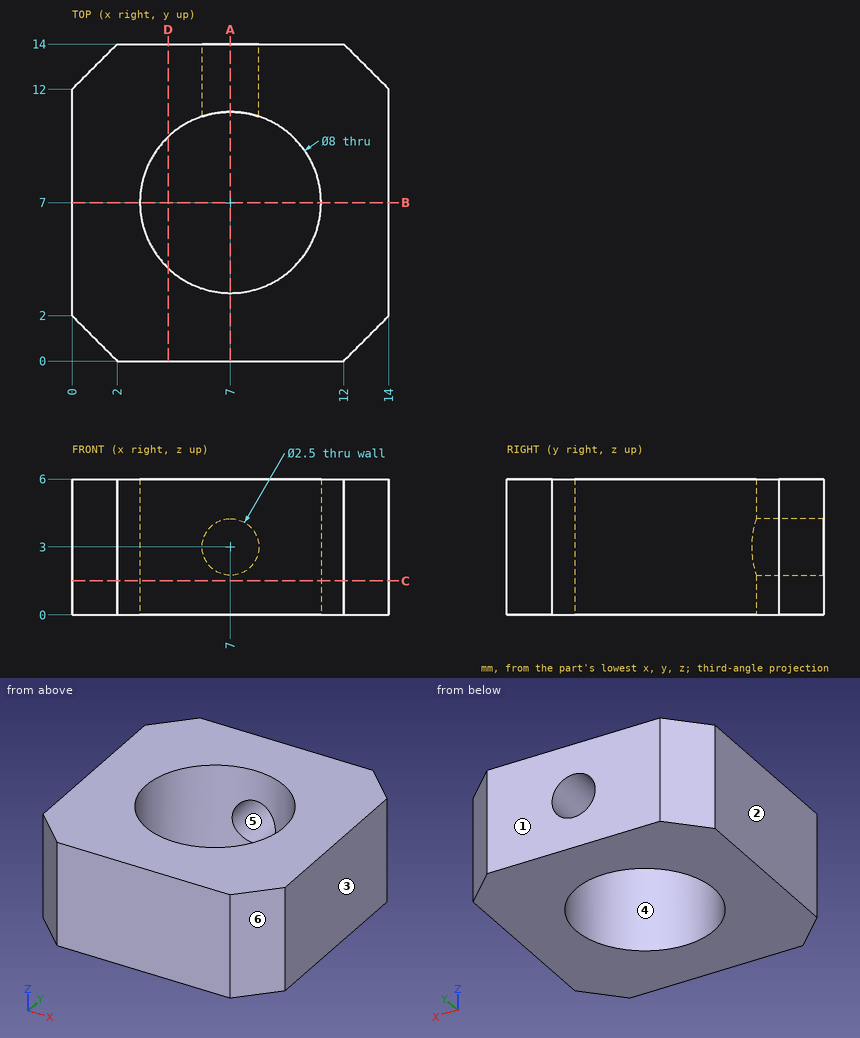
The drawing under review shows one solid part. Ordinate dimensions are in mm from its lowest x, y, z. A direction names the side the tool comes from. Coordinates: 2 decimals unless noted, no trailing zeros. Order: outer loops, then holes, each group sorted by start corner. A loop starts at its lowest first (then second) coordinate and runs counter-clockwise, first axis right, second up. Notation, with made-up numbers: (14.5, 40.25) -> (38.5, 40.25) arc R18 cw to (38.5, 68.25) -> close; hole circle Ø9 at (71.25, -14). An arc over 180 degrees is marked (long way). Answer in a Markdown table with one row per item. Add a question column.
Item 1: Mouldability with a two-part tool opening along X and no side actions: class the marked faces 1, 2, 3 and 4 as +X half, -X half, draft (parallel to the pull), parting line (faces both ways), or undercut.
Item 2: We need section D-D on x = 4.25. Write out the cut boundary in (y, z), plus the area to 3 significant figures.
Item 3: Clearance check with a flat-ended pin moving along its axis: pin 1 (2 mm diameter, centred on x = 9.5, z = 2.5, fed in from -Y). State where the tip first meets the part, or that it passes through.
Item 4: We need section B-B on y = 7. Write out the cut boundary in (x, z).
Item 5: We need section C-C on z = 1.5. Write out the cut boundary in (x, y).
Item 6: Machinability: for the marked faces 5 and 6, which of the approach directions +Z, -Z, +X, -X, +Y, -Y give a long, thin tool a straight path to every point of the face, cutting with its end or side? Answer none if there is none.
Item 7: To check wall thickness, follow probe 1 along Z at (x, y) = (7, 13.3); probe 2 along Y at (x, z) = (7, 1.5); probe 3 along X at (y, z) = (4.5, 5.25). State the ranges of each line that lie inside material, in increasing order.
Item 8: We need section A-A on x = 7. Write out the cut boundary in (y, z), plus the area to 3 significant figures.
Final values:
| question | item | result |
|---|---|---|
| 1 | face 1 | draft |
| 1 | face 2 | -X half |
| 1 | face 3 | +X half |
| 1 | face 4 | undercut |
| 2 | outline | (0, 0) -> (4.1, 0) -> (4.1, 6) -> (0, 6) -> close; (9.9, 0) -> (14, 0) -> (14, 6) -> (9.9, 6) -> close |
| 2 | area | 49.1 mm2 |
| 3 | pin 1 | stops at y = 0 |
| 4 | outline | (0, 0) -> (3, 0) -> (3, 6) -> (0, 6) -> close; (11, 0) -> (14, 0) -> (14, 6) -> (11, 6) -> close |
| 5 | outline | (0, 2) -> (2, 0) -> (12, 0) -> (14, 2) -> (14, 12) -> (12, 14) -> (2, 14) -> (0, 12) -> close; hole circle Ø8 at (7, 7) |
| 6 | face 5 | +Y |
| 6 | face 6 | +Z, -Z, +X, -Y |
| 7 | probe 1 | z = 0 to 1.75, 4.25 to 6 |
| 7 | probe 2 | y = 0 to 3, 11 to 14 |
| 7 | probe 3 | x = 0 to 3.88, 10.12 to 14 |
| 8 | outline | (0, 0) -> (3, 0) -> (3, 6) -> (0, 6) -> close; (11, 0) -> (14, 0) -> (14, 1.75) -> (11, 1.75) -> close; (11, 4.25) -> (14, 4.25) -> (14, 6) -> (11, 6) -> close |
| 8 | area | 28.5 mm2 |
